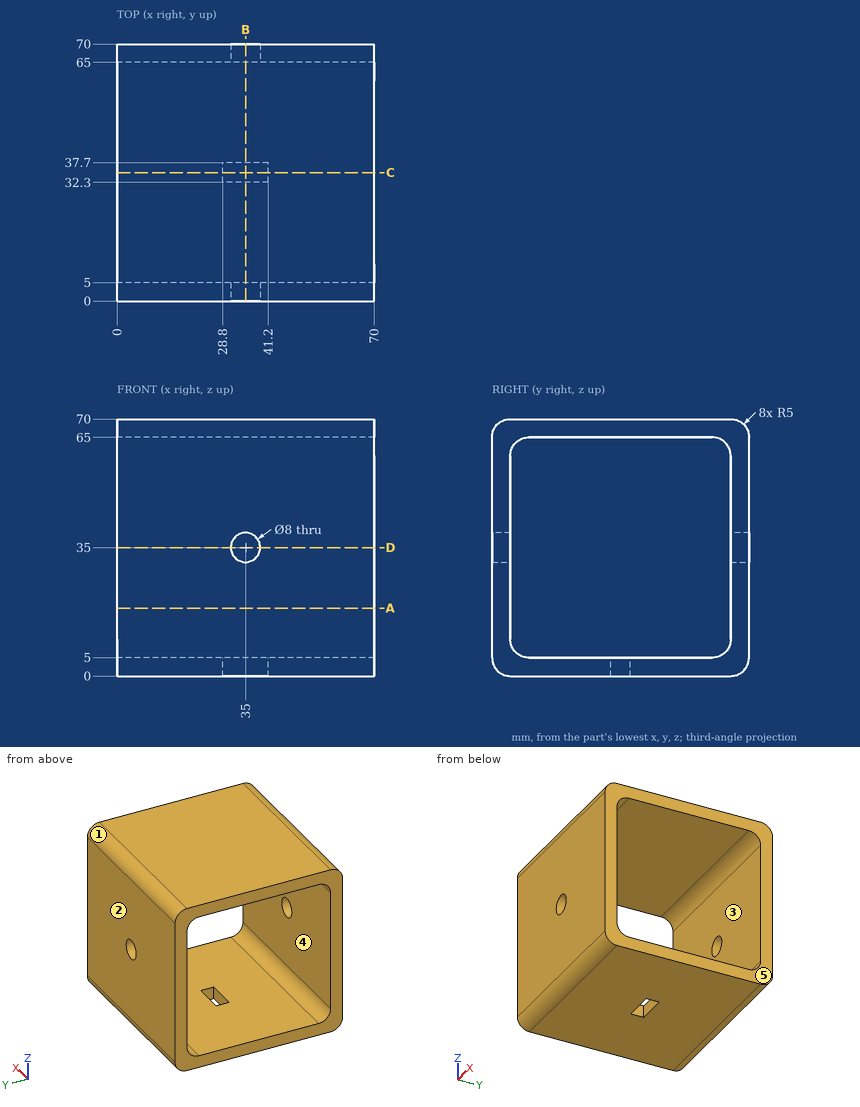
Can you work these out from the drawing? Everything is in mm from the part's minimum corner. A direction names the side the tool comes from. Round coordinates to 2 decimals unless told otherwise and drop trailing zeros. Order: outer loops, then holes, each group sorted by start corner. A loop starts at its lowest first (then second) coordinate and runs counter-clockwise, first axis right, second up. Notation, with made-up numbers: M -13.5,11 L 40.5,11 A14 ccw 40.5,19 Z; hole C 6.5,81.5 d9. An arc over 180 degrees is marked long. Answer as CSV lines item,"result".
Item 1: Imagine slicing it at B-B on x = 35. List the corners of the cut face in (y, z) for me.
From the geometry:
outline,"M 0,5 A5 ccw 5,0 L 32.3,0 L 32.3,5 L 10,5 A5 cw 5,10 L 5,31 L 0,31 Z; M 0,39 L 5,39 L 5,60 A5 cw 10,65 L 60,65 A5 cw 65,60 L 65,39 L 70,39 L 70,65 A5 ccw 65,70 L 5,70 A5 ccw 0,65 Z; M 37.7,0 L 65,0 A5 ccw 70,5 L 70,31 L 65,31 L 65,10 A5 cw 60,5 L 37.7,5 Z"
Item 2: Please list where these lines run through material, in increasing order: L1, parallel to Z at x = 22.5, y = 49.5; L2, parallel to X at y = 3, z = 35. Write a range as [from, to].
From the geometry:
L1,"[0, 5], [65, 70]"
L2,"[0, 31], [39, 70]"
Item 3: Imagine slicing it at A-A on z = 18.5. List the corners of the cut face in (x, y) for me, and give its area (3 significant figures).
From the geometry:
outline,"M 0,0 L 70,0 L 70,5 L 0,5 Z; M 0,65 L 70,65 L 70,70 L 0,70 Z"
area,"700 mm2"
Item 4: Imagine slicing it at D-D on z = 35. List the corners of the cut face in (x, y) for me.
From the geometry:
outline,"M 0,0 L 31,0 L 31,5 L 0,5 Z; M 0,65 L 31,65 L 31,70 L 0,70 Z; M 39,0 L 70,0 L 70,5 L 39,5 Z; M 39,65 L 70,65 L 70,70 L 39,70 Z"
Item 5: Which directions (+Z, -Z, +X, -X, +Y, -Y) give clear straight access to the entire face, cutting with the end or side of a thin tool? Please do the marked faces 4 and 5.
From the geometry:
face 4,"+X, -X"
face 5,"+Z, -Z, +X, +Y, -Y"
Item 6: For pin 1 (4 mm diameter, centred on x = 35.5, z = 3.5, fed in from -Y), with a flat end and sliding along its axis, tell me the tip position at first contact or that it passes through.
From the geometry:
pin 1,"y = 0"
Item 7: We'd pull the mould along Z, two halves only. Please class the marked faces 1, 2 and 3: +Z half, -Z half, draft (parallel to the pull), parting line (faces both ways), or undercut.
From the geometry:
face 1,"+Z half"
face 2,"draft"
face 3,"undercut"
Item 8: Imagine slicing it at C-C on y = 35. List the corners of the cut face in (x, z) for me, and give its area (3 significant figures).
From the geometry:
outline,"M 0,0 L 28.8,0 L 28.8,5 L 0,5 Z; M 0,65 L 70,65 L 70,70 L 0,70 Z; M 41.2,0 L 70,0 L 70,5 L 41.2,5 Z"
area,"638 mm2"
